```python
from build123d import *

# Parameters (mm, degrees)
HALF_SHELL_BODY_DEPTH   = 55
END_FLANGE_B_95X8_DEPTH = 8
END_START               = 8
END_FLANGE_A_95X8_DEPTH = 8
BORE_SKETCH_60_R        = 30
BORE_CUT_60_DEPTH       = 100


with BuildPart() as part:
    # Half Shell Profile Sketch → Half Shell Body (new, symmetric)
    with BuildSketch(Plane(origin=(0, 0, 0), x_dir=(0, 0, -1), z_dir=(1, 0, 0))):
        with BuildLine():
            Line((0, 39.686269666), (0, -39.686269666))
            ThreePointArc((0, -39.686269666), (45, 0), (0, 39.686269666))
        make_face()
    extrude(amount=HALF_SHELL_BODY_DEPTH, both=True)

    # End Flange B Sketch Ø95 → End Flange B Ø95x8 (add)
    with BuildSketch(Plane(origin=(55, 0, 0), x_dir=(0, 0, -1), z_dir=(1, 0, 0))):
        with BuildLine():
            Line((0, 47.236109069), (0, -47.236109069))
            ThreePointArc((0, -47.236109069), (52.5, 0), (0, 47.236109069))
        make_face()
    extrude(amount=END_FLANGE_B_95X8_DEPTH)

    # End Flange A Sketch Ø95 → End Flange A Ø95x8 (add)
    with BuildSketch(Plane.ZY.offset(55).offset(END_START)):
        with BuildLine():
            Line((0, 47.236109069), (0, -47.236109069))
            ThreePointArc((0, -47.236109069), (-52.5, 0), (0, 47.236109069))
        make_face()
    extrude(amount=-END_FLANGE_A_95X8_DEPTH)

    # Bore Sketch Ø60 → Bore Cut Ø60 (cut, symmetric)
    with BuildSketch(Plane(origin=(0, 0, 0), x_dir=(0, 0, -1), z_dir=(1, 0, 0))):
        with Locations((5, 0)):
            Circle(BORE_SKETCH_60_R)
    extrude(amount=BORE_CUT_60_DEPTH, both=True, mode=Mode.SUBTRACT)


solid = part.part
```
Work out the finished part from the listing and answer in its coordinate system (mm). Coordinates: 2 decimals unless noted, no trailing zeros. Loops run counter-clockwise (first coordinate to the right, second up) from the corner with the lowest first, then second, coordinate; pieces in that order, holes last. Notation, with made-up numbers: M 70.5,82.25 L 78.5,82.25 A33 cw 78.5,114.25 Z; hole C 3.5,-15 d11. An arc over 180 degrees is marked long. Use CSV: the item, a comma, the result in double quotes. Start each with the question number.
(1) Given pin 1 Ø1 at (x, y) = (29.5, -30.5) entering from -Z; pin 2 Ø8 at (x, z) = (-27.5, -25.5) entering from +Y; pin 3 Ø6 at (x, y) = (-15, 4) entering from +Z; pin 4 Ø3 at (y, z) = (28, -46) entering from +X, each flat-ended and moving along its own axis, determine where each tip first touches the part or whether it passes through.
(2) Consider line 1 (X direction, y = 23, z = -45); line 2 (Y direction, x = 31, z = -5); line 3 (Y direction, x = -0.5, z = -8). Determine where each line is inside the solid, lowest interval first.
(3) Find section C-C, the plane z = -42. Give the vertices of the cut face in (x, y).
(4) Find section B-B, the plane y = 0. Give the vertices of the cut face in (x, z), then the cut area to 3 significant figures.
(5) For a pull along Z with two mould halves and no side action, classify faces 1 (the face through (55, 4, -46)), 2 (the face through (-1, 37, 0)), 3 (the face through (0.88, -0.73, -34.99)) as +Z half, -Z half, draft (parallel to the pull), parting line (faces both ways), or undercut.
(6) Find section A-A, the plane z = -5. Give the vertices of the cut face in (x, y).
(7) Find section D-D, the plane x = 19. Give the vertices of the cut face in (y, z), then the cut area to 3 significant figures.
Recorded:
1,pin 1,"stops at z = -31.46"
1,pin 2,"stops at y = 36.44"
1,pin 3,"stops at z = -34.17"
1,pin 4,"passes through"
2,line 1,"x = -63 to -55, 55 to 63"
2,line 2,"y = -40 to -30, 30 to 40"
2,line 3,"y = -39.89 to -29.85, 29.85 to 39.89"
3,outline,"M -63,-29.79 L -55,-29.79 L -55,-15.2 L 55,-15.2 L 55,-29.79 L 63,-29.79 L 63,29.79 L 55,29.79 L 55,15.2 L -55,15.2 L -55,29.79 L -63,29.79 Z"
4,outline,"M -63,-52.5 L -55,-52.5 L -55,-45 L 55,-45 L 55,-52.5 L 63,-52.5 L 63,-35 L -63,-35 Z"
4,area,"1,380 mm^2"
5,face 1,"draft"
5,face 2,"+Z half"
5,face 3,"undercut"
6,outline,"M -63,-47.5 L -55,-47.5 L -55,-40 L 55,-40 L 55,-47.5 L 63,-47.5 L 63,-30 L -63,-30 Z; M -63,30 L 63,30 L 63,47.5 L 55,47.5 L 55,40 L -55,40 L -55,47.5 L -63,47.5 Z"
7,outline,"M -39.69,0 A40 ccw long 39.69,0 L 29.58,0 A30 cw long -29.58,0 Z"
7,area,"1,200 mm^2"
